Verification items for the finished model (mm, model axes). A direction names the side the tool comes from. Coordinates: 2 decimals unless noted, no trailing zeros. Order: outer loops, then holes, each group sorted by start corner. A loop starts at its lowest first (then second) coordinate and runs counter-clockwise, first axis right, second up. Notation, with made-up numbers: M -8,-25 L 40,-25 A20 cw 40,-14 Z; hole C 76,-36.5 d6. An arc over 180 degrees is marked long. Return JSON: item names as keys, results as strings. Group by question number.
1. Section check A-A, the plane z = 5.75. Give the number of separate pieces and of enclosed holes in the cut face, plus the area to 3 significant figures.
2. Material ranges on line 1 along Y through (x, z) = (22.5, 4.5); line 2 along X through (y, z) = (-1, 18); line 3 along Z through (x, y) = (30, -15), recorded low to high.
3. Section check B-B, the plane x = 18. Record the cut outline in (y, z), plus the area to 3 significant figures.
4. Section check C-C, the plane z = 15. Record the cut outline in (x, y), plus the area to 3 significant figures.
5. Set-up check for faces 4 (the flat face through (11, 7.6, 19)), 5 (the flat face through (12, -11, 11)), 6 (the cylindrical face through (21, -15, 5)): record each of +Z, -Z, +X, -X, +Y, -Y from which the full face is reachable in a straight line by a thin tool's end or side.
6. Mould release check, pull along X, two halves, no side actions. Record for faces 1 (the cylindrical face through (-0.54, 10.56, 5.07)), 2 (the cylindrical face through (30.1, 0.17, 18.9)), 3 (the flat face through (12, 0, 0)): +X half, -X half, draft (parallel to the pull), parting line (faces both ways), or undercut.
7. Gauge pin test, flat ends, axial feed: pin 1 (6 mm diameter, centred on y = -1.5, z = 12.5, fed in from -X); pin 2 (4 mm diameter, centred on x = 23, z = 18, fed in from -Y); pin 3 (7.5 mm diameter, centred on x = 36.5, y = -0.5, fed in from +Z). Record the tip position at first contact, or that the pin passes through.
```python
from build123d import *

# Parameters (mm, degrees)
BASE_FLANGE_DEPTH          = 11
OBROUND_BOSS_DEPTH         = 15
BOSS_POCKET_DEPTH          = 5
MOUNTING_HOLES_A_PROFILE_R = 2.5
MOUNTING_HOLES_A_DEPTH     = 47.789421881
SPOT_FACES_A_PROFILE_R     = 3.5
SPOT_FACES_A_DEPTH         = 1
CENTRE_HOLES_PROFILE_R     = 2.5
CENTRE_HOLES_DEPTH         = 50.043348173
BOSS_ROOT_FILLET_R1_R      = 1
MOUNTING_HOLES_B_PROFILE_R = 2.5
MOUNTING_HOLES_B_DEPTH     = 47.789421881
SPOT_FACES_B_PROFILE_R     = 3.5
SPOT_FACES_B_DEPTH         = 1


with BuildPart() as part:
    # Flange Profile → Base Flange (new body)
    with BuildSketch(Plane.XY):
        with BuildLine():
            Line((0, 18), (22.5, 18))
            ThreePointArc((22.5, 18), (40.5, 0), (22.5, -18))
            Line((22.5, -18), (0, -18))
            ThreePointArc((0, -18), (-18, 0), (0, 18))
        make_face()
    extrude(amount=BASE_FLANGE_DEPTH)

    # Boss Profile → Obround Boss (add)
    with BuildSketch(Plane.XY.offset(11)):
        with BuildLine():
            Line((0, 7.6), (22.5, 7.6))
            ThreePointArc((22.5, 7.6), (30.1, 0), (22.5, -7.6))
            Line((22.5, -7.6), (0, -7.6))
            ThreePointArc((0, -7.6), (-7.6, 0), (0, 7.6))
        make_face()
    extrude(amount=OBROUND_BOSS_DEPTH)

    # Boss Pocket Profile → Boss Pocket (cut)
    with BuildSketch(Plane.XY.offset(26)):
        with BuildLine():
            Line((0, 5), (22.5, 5))
            ThreePointArc((22.5, 5), (27.5, 0), (22.5, -5))
            Line((22.5, -5), (0, -5))
            ThreePointArc((0, -5), (-5, 0), (0, 5))
        make_face()
    extrude(amount=-BOSS_POCKET_DEPTH, mode=Mode.SUBTRACT)

    # Mounting Holes A Profile → Mounting Holes A (cut, through all)
    with BuildSketch(Plane.XY.offset(11)):
        with Locations((0, 13)):
            Circle(MOUNTING_HOLES_A_PROFILE_R)
        with Locations((22.5, 13)):
            Circle(MOUNTING_HOLES_A_PROFILE_R)
        with Locations((0, -13)):
            Circle(MOUNTING_HOLES_A_PROFILE_R)
        with Locations((22.5, -13)):
            Circle(MOUNTING_HOLES_A_PROFILE_R)
    extrude(amount=-MOUNTING_HOLES_A_DEPTH, mode=Mode.SUBTRACT)

    # Spot Faces A Profile → Spot Faces A (cut)
    with BuildSketch(Plane.XY.offset(11)):
        with Locations((0, 13)):
            Circle(SPOT_FACES_A_PROFILE_R)
        with Locations((22.5, 13)):
            Circle(SPOT_FACES_A_PROFILE_R)
        with Locations((22.5, -13)):
            Circle(SPOT_FACES_A_PROFILE_R)
        with Locations((0, -13)):
            Circle(SPOT_FACES_A_PROFILE_R)
    extrude(amount=-SPOT_FACES_A_DEPTH, mode=Mode.SUBTRACT)

    # Centre Holes Profile → Centre Holes (cut, through all)
    with BuildSketch(Plane.XY.offset(21)):
        Circle(CENTRE_HOLES_PROFILE_R)
        with Locations((22.50803184, 0)):
            Circle(CENTRE_HOLES_PROFILE_R)
    extrude(amount=-CENTRE_HOLES_DEPTH, mode=Mode.SUBTRACT)

    # Boss Root Fillet R1
    boss_root_fillet_r1_edges = [part.edges().sort_by_distance(p)[0] for p in [
        (40.5, 0, 11),
        (-7.6, 0, 11),
        (11.25, -7.6, 11),
        (11.25, 18, 11),
        (30.1, 0, 11),
        (11.25, 7.6, 11),
        (-18, 0, 11),
        (11.25, -18, 11),
    ]]
    fillet(boss_root_fillet_r1_edges, radius=BOSS_ROOT_FILLET_R1_R)

    # Mounting Holes B Profile → Mounting Holes B (cut, through all)
    with BuildSketch(Plane.XY.offset(11)):
        with Locations((-13, 0)):
            Circle(MOUNTING_HOLES_B_PROFILE_R)
        with Locations((35.50803184, 0)):
            Circle(MOUNTING_HOLES_B_PROFILE_R)
    extrude(amount=-MOUNTING_HOLES_B_DEPTH, mode=Mode.SUBTRACT)

    # Spot Faces B Profile → Spot Faces B (cut)
    with BuildSketch(Plane.XY.offset(11)):
        with Locations((-13, 0)):
            Circle(SPOT_FACES_B_PROFILE_R)
        with Locations((35.50803184, 0)):
            Circle(SPOT_FACES_B_PROFILE_R)
    extrude(amount=-SPOT_FACES_B_DEPTH, mode=Mode.SUBTRACT)


solid = part.part
```
Answers follow:
{
 "1": {"separate pieces": "1", "enclosed holes": "8", "area": "1,670 mm^2"},
 "2": {"line 1": "-18 to -15.5, -10.5 to -2.5, 2.5 to 10.5, 15.5 to 18", "line 2": "-7.53 to -2.29, 2.29 to 20.22, 24.8 to 30.03", "line 3": "0 to 11"},
 "3": {"outline": "M -18,0 L 18,0 L 18,10 A1 ccw 17,11 L 8.6,11 A1 cw 7.6,12 L 7.6,26 L 5,26 L 5,21 L -5,21 L -5,26 L -7.6,26 L -7.6,12 A1 cw -8.6,11 L -17,11 A1 ccw -18,10 Z", "area": "574 mm^2"},
 "4": {"outline": "M 0,-7.6 L 22.5,-7.6 A7.6 ccw 22.5,7.6 L 0,7.6 A7.6 ccw Z; hole C 0,0 d5; hole C 22.51,0 d5", "area": "484 mm^2"},
 "5": {"face 4": "+Z, +X, -X, +Y", "face 5": "+Z", "face 6": "+Z, -Z"},
 "6": {"face 1": "undercut", "face 2": "+X half", "face 3": "draft"},
 "7": {"pin 1": "x = -18", "pin 2": "y = -7.6", "pin 3": "z = 11"}
}
